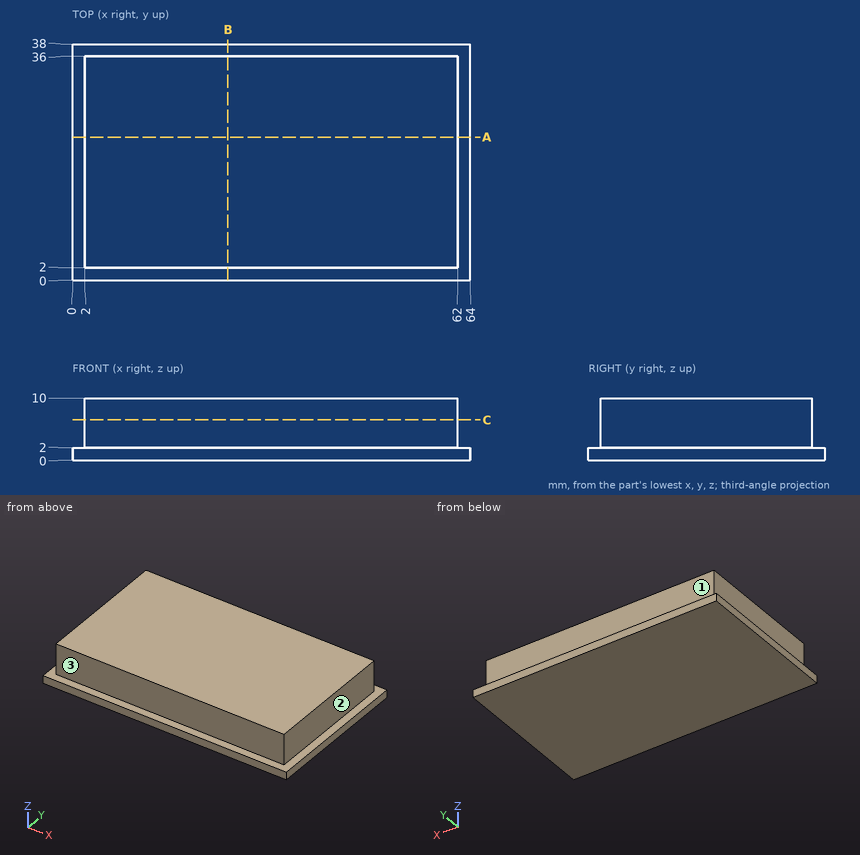
Can you work these out from the drawing? Everything is in mm from the part's minimum corner. A direction names the side the tool comes from. Give positions to 0.01 mm unless a question says otherwise; leave off trailing zeros. Order: outer loops, then holes, each group sorted by start corner. A loop starts at its lowest first (then second) coordinate and runs counter-clockwise, first axis right, second up. Notation, with made-up numbers: M 18.5,35.5 L 27.5,35.5 A13 cw 27.5,45.5 Z; hole C -28,57 d11. An arc over 180 degrees is marked long. Write item = value, one per line. Start each with the question number.
Q1. I need wall thicknesses on probe 1 along Y at (x, z) = (36.5, 9.75); probe 2 along X at (y, z) = (35.5, 4.5). Which ranges of each line are inside material? Lowest first, please. Write a range as [from, to].
Q2. For the marked faces 1, 2 and 3, which set-ups out of +Z, -Z, +X, -X, +Y, -Y let a thin tool reach every point of the face, with its end or its side?
Q3. Suppose I cut it at B-B (x = 25). Write out the boundary of the cut face in (y, z).
Q4. Suppose I cut it at C-C (z = 6.5). Write out the boundary of the cut face in (x, y).
Q5. Suppose I cut it at A-A (y = 23). Write out the boundary of the cut face in (x, z), plus the area to 3 significant figures.
Q6. Will these pins go through, and if not, where does the flat tip stop? pin 1 Ø4 at (y, z) = (23, 5) entering from +X; pin 2 Ø3 at (x, z) = (45, 5.5) entering from -Y.
Check result:
q1.probe_1 = [2, 36]
q1.probe_2 = [2, 62]
q2.face_1 = +Z, +X, -X, +Y
q2.face_2 = +Z, +X, +Y, -Y
q2.face_3 = +Z, +X, -X, -Y
q3.outline = M 0,0 L 38,0 L 38,2 L 36,2 L 36,10 L 2,10 L 2,2 L 0,2 Z
q4.outline = M 2,2 L 62,2 L 62,36 L 2,36 Z
q5.outline = M 0,0 L 64,0 L 64,2 L 62,2 L 62,10 L 2,10 L 2,2 L 0,2 Z
q5.area = 608 mm2
q6.pin_1 = 62
q6.pin_2 = 2
